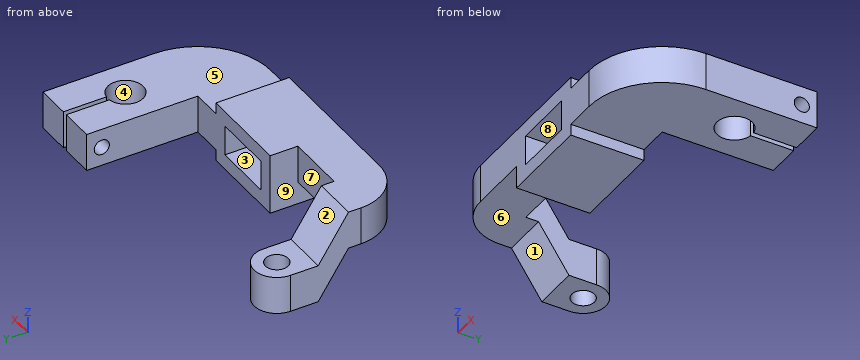
```python
from build123d import *

# Parameters (mm, degrees)
BRACKET_BODY_DEPTH         = 12
BODY_RELIEF_CUT_DEPTH      = 75.57211275
BODY_RELIEF_CUT_DEPTH_BACK = 75.57211275
BODY_RELIEF_SKETCH_W       = 24
BODY_RELIEF_SKETCH_H       = 12
BODY_RELIEF_SKETCH_H_2     = 9
BODY_RELIEF_SKETCH_W_2     = 41
BODY_RELIEF_SKETCH_H_3     = 4.5
RECTANGULAR_WINDOW_DEPTH   = 86.343423883
CLAMP_HOLE_SKETCH_R        = 3
CLAMP_HOLE_6_DEPTH         = 94.542770966
ARM_BOSS_DEPTH             = 15
PIVOT_LUG_DEPTH            = 18
LUG_FILL_BOSS_DEPTH        = 15
PIVOT_BORE_SKETCH_R        = 4.5
PIVOT_BORE_9_DEPTH         = 24


with BuildPart() as part:
    # Bracket Profile Sketch → Bracket Body (new, symmetric)
    with BuildSketch(Plane.XY):
        with BuildLine():
            Line((30, 14.5), (30, 58.5))
            Line((30, 58.5), (59, 58.5))
            Line((59, 58.5), (59, 14.5))
            ThreePointArc((59, 14.5), (50.506096654, -6.006096654), (30, -14.5))
            Line((30, -14.5), (18, -14.5))
            Line((18, -14.5), (-18, -14.5))
            Line((-18, -14.5), (-42, -14.5))
            Line((-42, -14.5), (-42, 3.5))
            Line((-42, 3.5), (-18, 3.5))
            Line((-18, 3.5), (-18, 14.5))
            Line((-18, 14.5), (18, 14.5))
            Line((18, 14.5), (30, 14.5))
        make_face()
    extrude(amount=BRACKET_BODY_DEPTH, both=True)

    # Body Relief Sketch → Body Relief Cut (cut, two sides: drawn at the far end of the back side and taken through both)
    with BuildSketch(Plane(origin=(0, 14.5, 0), x_dir=(1, 0, 0), z_dir=(0, 1, 0)).offset(-BODY_RELIEF_CUT_DEPTH_BACK)):
        Rectangle(BODY_RELIEF_SKETCH_W, BODY_RELIEF_SKETCH_H)
        with Locations((-30, 7.5)):
            Rectangle(BODY_RELIEF_SKETCH_W, BODY_RELIEF_SKETCH_H_2)
        with Locations((38.5, -9.75)):
            Rectangle(BODY_RELIEF_SKETCH_W_2, BODY_RELIEF_SKETCH_H_3)
        with Locations((38.5, 9.75)):
            Rectangle(BODY_RELIEF_SKETCH_W_2, BODY_RELIEF_SKETCH_H_3)
    extrude(amount=BODY_RELIEF_CUT_DEPTH + BODY_RELIEF_CUT_DEPTH_BACK, mode=Mode.SUBTRACT)

    # Window Sketch → Rectangular Window (cut, through all)
    with BuildSketch(Plane.XY.offset(7.5)):
        with BuildLine():
            Line((43.5, 41.42820323), (43.5, 58.5))
            Line((43.5, 58.5), (45.5, 58.5))
            Line((45.5, 58.5), (45.5, 41.42820323))
            ThreePointArc((45.5, 41.42820323), (44.5, 27.5), (43.5, 41.42820323))
        make_face()
    extrude(amount=-RECTANGULAR_WINDOW_DEPTH, mode=Mode.SUBTRACT)

    # Clamp Hole Sketch → Clamp Hole Ø6 (cut, through all)
    with BuildSketch(Plane.ZY.offset(-30)):
        with Locations((0, 52.5)):
            Circle(CLAMP_HOLE_SKETCH_R)
    extrude(amount=-CLAMP_HOLE_6_DEPTH, mode=Mode.SUBTRACT)

    # Arm Sketch → Arm Boss (add)
    with BuildSketch(Plane.XY.offset(12)):
        with BuildLine():
            Line((-60, 3.5), (-60, 8.5))
            Line((-60, 8.5), (-42, 8.5))
            Line((-42, 8.5), (-42, 3.5))
            Line((-42, 3.5), (-42, -14.5))
            ThreePointArc((-42, -14.5), (-54.727922061, -9.227922061), (-60, 3.5))
        make_face()
    extrude(amount=-ARM_BOSS_DEPTH)

    # Pivot Lug Sketch → Pivot Lug (add)
    with BuildSketch(Plane.ZY.offset(60)):
        Polygon((-3, 8.5), (-21, 20.5), (-21, 31.5), (-6, 31.5), (-6, 20.5), (12, 8.5), align=None)
    extrude(amount=-PIVOT_LUG_DEPTH)

    # Lug Fill Sketch → Lug Fill Boss (add)
    with BuildSketch(Plane.XY.offset(-6)):
        with BuildLine():
            Line((-60, 31.5), (-42, 31.5))
            ThreePointArc((-42, 31.5), (-51, 40.5), (-60, 31.5))
        make_face()
    extrude(amount=-LUG_FILL_BOSS_DEPTH)

    # Pivot Bore Sketch → Pivot Bore Ø9 (cut)
    with BuildSketch(Plane.XY.offset(-6)):
        with Locations((-51, 31.5)):
            Circle(PIVOT_BORE_SKETCH_R)
    extrude(amount=-PIVOT_BORE_9_DEPTH, mode=Mode.SUBTRACT)


solid = part.part
```
Model file for the job. Use its own axes, mm. Face numbers are marked on the shaded views. A direction names the side the tool comes from. Coordinates: 2 decimals unless noted, no trailing zeros. Write each loop counter-clockwise with the first axis right and the second up, starting at its lowest first coordinate (ties: lowest second). Pieces come first, ordered by that corner, then holes. Notation, with made-up numbers: (-19.5, -5) - (39.5, -5) arc R29 cw to (39.5, 22) - close; hole circle Ø6 at (81, 67.25). An arc over 180 degrees is marked (long way). One line per question, with ' | ' between items. Start each with the question number.
Q1. Pull direction Z, two halves, no side cores. Call the marked faces 1, 2, 3 and 4: pulls with the +Z half, pulls with the -Z half, needs draft (parallel to the pull), parting line crosses it, or undercut.
Q2. 3-axis set-ups, long thin cutter, end or side, ignore diameter. For the marked faces 5, 6, 7, 8 and 9: which of +Z, -Z, +X, -X, +Y, -Y reach the whole face in a straight line?
Q3. Pin check, flat tips, straight feed: pin 1 (9.5 mm diameter, centred on y = 52.5, z = 0, fed in from +X); pin 2 (14.5 mm diameter, centred on x = 5.5, y = -5.5, fed in from -Z); pin 3 (3 mm diameter, centred on x = 37.5, y = 4.5, fed in from +Z); pin 4 (5 mm diameter, centred on y = -3, z = 10.5, fed in from +X). Stop position of each tip, or through.
Q4. Cut at C-C, the plane z = 0. List the corners of the cut face in (x, y).
Q5. Drill centre lines: line 1 (X direction, y = 4, z = 10.5); line 2 (X direction, y = 34, z = 2); line 3 (Z direction, x = -6.5, y = 8). Where is each one in solid material? Low to high. Write a range as [from, to].
Q6. Cut at B-B, the plane y = 43. List the corners of the cut face in (x, z), then the cut area to 3 significant figures.
Q7. Cut at D-D, the plane x = 47.5. List the corners of the cut face in (y, z), then the cut area to 3 significant figures.
Q8. Cut at A-A, the plane y = 52.5. List the corners of the cut face in (x, z).
Answer below:
1) face 1: pulls with the -Z half | face 2: pulls with the +Z half | face 3: undercut | face 4: needs draft
2) face 5: +Z, +X, +Y, -Y | face 6: -Z, -X, -Y | face 7: +Z, -Z, +Y | face 8: +Y, -Y | face 9: -Z, +Y
3) pin 1: x = 59 | pin 2: z = -12 | pin 3: z = 7.5 | pin 4: x = 18
4) outline: (-60, 3.5) arc R18 ccw to (-42, -14.5) - (-12, -14.5) - (-12, 14.5) - (-18, 14.5) - (-18, 3.5) - (-42, 3.5) - (-42, 16.5) - (-60, 16.5) - close; (12, -14.5) - (30, -14.5) arc R29 ccw to (59, 14.5) - (59, 49.5) - (45.5, 49.5) - (45.5, 41.43) arc R7 cw (long way) to (43.5, 41.43) - (43.5, 49.5) - (30, 49.5) - (30, 14.5) - (12, 14.5) - close; (30, 55.5) - (43.5, 55.5) - (43.5, 58.5) - (30, 58.5) - close; (45.5, 55.5) - (59, 55.5) - (59, 58.5) - (45.5, 58.5) - close
5) line 1: [-60, -42], [-18, 18] | line 2: [30, 37.52], [51.48, 59] | line 3: [-12, -6], [6, 12]
6) outline: (30, -7.5) - (43.5, -7.5) - (43.5, 7.5) - (30, 7.5) - close; (45.5, -7.5) - (59, -7.5) - (59, 7.5) - (45.5, 7.5) - close | area: 405 mm^2
7) outline: (-8.62, -7.5) - (28.18, -7.5) - (28.18, 7.5) - (-8.62, 7.5) - close; (40.82, -7.5) - (58.5, -7.5) - (58.5, 7.5) - (40.82, 7.5) - close; hole circle Ø6 at (52.5, 0) | area: 789 mm^2
8) outline: (30, -7.5) - (43.5, -7.5) - (43.5, -3) - (30, -3) - close; (30, 3) - (43.5, 3) - (43.5, 7.5) - (30, 7.5) - close; (45.5, -7.5) - (59, -7.5) - (59, -3) - (45.5, -3) - close; (45.5, 3) - (59, 3) - (59, 7.5) - (45.5, 7.5) - close
